Check sheet for the modelled part. Datum: model origin and axes. Units: mm. Face numbers are marked on the shaded views. A direction names the side the tool comes from. Coordinates: 2 decimals unless noted, no trailing zeros. Write each loop counter-clockwise with the first axis right and the second up, starting at its lowest first coordinate (ties: lowest second). Pieces come first, ordered by that corner, then holes. Notation, with made-up numbers: (72.25, -8.75) -> (119.25, -8.75) arc R19 cw to (119.25, 17.25) -> close; hole circle Ø9 at (63.25, -10.75). An arc over 180 degrees is marked (long way). One line per item, written item: value. Start each with the question number.
1) Sectioned sample at C-C on z = 43.5. Enter the section's corners in (x, y), plus the area to 3 significant figures.
2) Scan lines: line 1 along X through (y, z) = (-77.75, 25); line 2 along X through (y, z) = (-19.5, 33); line 3 along X through (y, z) = (-75, 25). Record each from-to range of solid material in increasing order. Write a range as [from, to].
3) Draft check along X on the marked faces 3, 4, 5 and 6. Enter one of: +X half, -X half, draft (parallel to the pull), parting line (faces both ways), or undercut.
4) Set-up check for the marked faces 1 and 2: record each of +Z, -Z, +X, -X, +Y, -Y from which the full face is reachable in a straight line by a thin tool's end or side.
5) Sectioned sample at A-A on x = 50. Enter the section's corners in (y, z).
6) Sectioned sample at D-D on z = 30.5. Enter the section's corners in (x, y).
7) Gauge pin test, flat end, axial feed: P1, Ø17, axis at x = 50, z = 25, coming from the +Y side. Record the tip position at first contact, or that the pin passes through.
8) Sectioned sample at B-B on z = 25. Enter the section's corners in (x, y), plus the area to 3 significant figures.
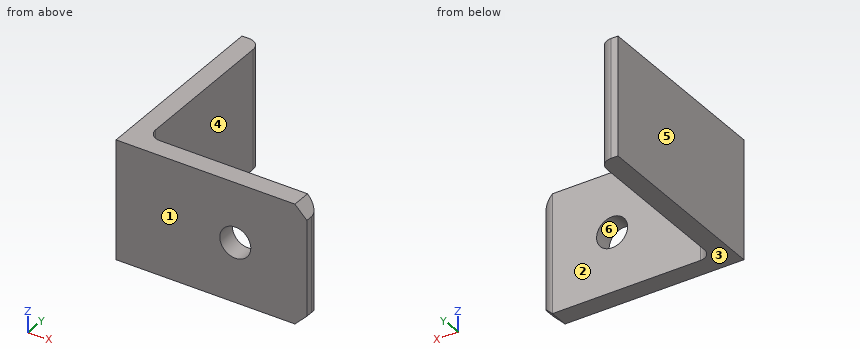
```python
from build123d import *

# Parameters (mm, degrees)
EXTRUDE_1_DEPTH     = 50
SKETCH_2_R          = 6.5
CUT_EXTRUDE_1_DEPTH = 50
FILLET_1_R          = 5
FILLET_2_R          = 5
CHAMFER_1_SIZE      = 5
FILLET_3_R          = 5


with BuildPart() as part:
    # 草图1 → 凸台-拉伸1 (new body)
    with BuildSketch(Plane.XY):
        Polygon((0, 0), (0, -80), (80, -80), (80, -72), (8, -72), (8, 0), align=None)
    extrude(amount=EXTRUDE_1_DEPTH)

    # 草图2 → 切除-拉伸1 (cut)
    with BuildSketch(Plane(origin=(0, -72, 0), x_dir=(1, 0, 0), z_dir=(0, 1, 0))):
        with Locations(Location((50, -25, 0), (0, 0, 270))):
            Circle(SKETCH_2_R)
    extrude(amount=-CUT_EXTRUDE_1_DEPTH, mode=Mode.SUBTRACT)

    # 圆角1
    fillet_1_edges = [part.edges().sort_by_distance(p)[0] for p in [
        (8, -72, 25),
    ]]
    fillet(fillet_1_edges, radius=FILLET_1_R)

    # 圆角2
    fillet_2_edges = [part.edges().sort_by_distance(p)[0] for p in [
        (8, 0, 25),
    ]]
    fillet(fillet_2_edges, radius=FILLET_2_R)

    # 倒角1
    chamfer_1_edges = [part.edges().sort_by_distance(p)[0] for p in [
        (80, -76, 0),
        (80, -76, 50),
    ]]
    chamfer(chamfer_1_edges, length=CHAMFER_1_SIZE)

    # 圆角3
    fillet_3_edges = [part.edges().sort_by_distance(p)[0] for p in [
        (80, -72, 25),
    ]]
    fillet(fillet_3_edges, radius=FILLET_3_R)


solid = part.part
```
Answers:
1. outline: (0, -80) -> (80, -80) -> (80, -77) arc R5 ccw to (75, -72) -> (13, -72) arc R5 cw to (8, -67) -> (8, -5) arc R5 ccw to (3, 0) -> (0, 0) -> close
1. area: 1,210 mm2
2. line 1: x = [0, 43.5], [56.5, 80]
2. line 2: x = [0, 8]
2. line 3: x = [0, 43.5], [56.5, 79.58]
3. face 3: draft
3. face 4: +X half
3. face 5: -X half
3. face 6: undercut
4. face 1: +Z, -Z, +X, -X, -Y
4. face 2: +Z, -Z, +X, +Y
5. outline: (-80, 0) -> (-72, 0) -> (-72, 18.5) -> (-80, 18.5) -> close; (-80, 31.5) -> (-72, 31.5) -> (-72, 50) -> (-80, 50) -> close
6. outline: (0, -80) -> (46.54, -80) -> (46.54, -72) -> (13, -72) arc R5 cw to (8, -67) -> (8, -5) arc R5 ccw to (3, 0) -> (0, 0) -> close; (53.46, -80) -> (80, -80) -> (80, -77) arc R5 ccw to (75, -72) -> (53.46, -72) -> close
7. P1: stops at y = -72
8. outline: (0, -80) -> (43.5, -80) -> (43.5, -72) -> (13, -72) arc R5 cw to (8, -67) -> (8, -5) arc R5 ccw to (3, 0) -> (0, 0) -> close; (56.5, -80) -> (80, -80) -> (80, -77) arc R5 ccw to (75, -72) -> (56.5, -72) -> close
8. area: 1,110 mm2
